CAD build for the part. Positions are in the model's coordinates, mm. A direction names the side the tool comes from. Give positions to 0.01 mm unless a question says otherwise; leave off trailing zeros. Write each loop counter-clockwise with the first axis right and the second up, starting at its lowest first coordinate (ties: lowest second). Pieces come first, ordered by that corner, then holes. Notation, with made-up numbers: (-14, 5.25) - (33, 5.25) arc R36 ccw to (33, 41.25) - close; hole circle Ø6 at (-5.5, -25.5). An arc over 180 degrees is marked (long way). Write item = value, one per line. Start each with the question number.
```python
from build123d import *

# Parameters (mm, degrees)
SKETCH3_OUTSIDE_W   = 136.718
SKETCH3_OUTSIDE_H   = 136.718
CUT_EXTRUDE2_DEPTH  = 5.463617
SKETCH4_W           = 9.6
SKETCH4_H           = 1.5
BOSS_EXTRUDE1_DEPTH = 6


with BuildPart() as part:
    # Sketch2 → Base-Revolve (revolve)
    with BuildSketch(Plane(origin=(0, 0, 0), x_dir=(0, 0, -1), z_dir=(1, 0, 0))):
        Polygon((-3.963615094, 52.5), (0, 44), (0, 0), (-1.5, 0), (-1.5, 44), (-5.463615094, 52.5), align=None)
    revolve(axis=Axis((0, 0, 0), (0, 0, 1)))

    # Sketch3 outside → Cut-Extrude2 (cut)
    # profile 1 of 2: a face of its own
    with BuildSketch(Plane.XY):
        Rectangle(SKETCH3_OUTSIDE_W, SKETCH3_OUTSIDE_H)
        with BuildLine():
            Line((-4.8, -43.737398185), (-4.8, -52.280110941))
            Line((-4.8, -52.280110941), (4.8, -52.280110941))
            Line((4.8, -52.280110941), (4.8, -43.737398185))
            ThreePointArc((4.8, -43.737398185), (34.907546973, -26.785502876), (43.489413898, 6.683627667))
            Line((43.489413898, 6.683627667), (51.741040776, 8.894644425))
            Line((51.741040776, 8.894644425), (49.256377943, 18.167532358))
            Line((49.256377943, 18.167532358), (41.004751065, 15.9565156))
            ThreePointArc((41.004751065, 15.9565156), (38.105117767, 22), (34.321123398, 27.532898298))
            Line((34.321123398, 27.532898298), (40.361733517, 33.573508418))
            Line((40.361733517, 33.573508418), (33.573508418, 40.361733517))
            Line((33.573508418, 40.361733517), (27.532898298, 34.321123398))
            ThreePointArc((27.532898298, 34.321123398), (22, 38.105117767), (15.9565156, 41.004751065))
            Line((15.9565156, 41.004751065), (18.167532358, 49.256377943))
            Line((18.167532358, 49.256377943), (8.894644425, 51.741040776))
            Line((8.894644425, 51.741040776), (6.683627667, 43.489413898))
            ThreePointArc((6.683627667, 43.489413898), (-34.907546973, 26.785502876), (-40.277697924, -17.711777154))
            Line((-40.277697924, -17.711777154), (-47.675904188, -21.983133532))
            Line((-47.675904188, -21.983133532), (-42.875904188, -30.296977409))
            Line((-42.875904188, -30.296977409), (-35.477697924, -26.025621031))
            ThreePointArc((-35.477697924, -26.025621031), (-31.112698372, -31.112698372), (-26.025621031, -35.477697924))
            Line((-26.025621031, -35.477697924), (-30.296977409, -42.875904188))
            Line((-30.296977409, -42.875904188), (-21.983133532, -47.675904188))
            Line((-21.983133532, -47.675904188), (-17.711777154, -40.277697924))
            ThreePointArc((-17.711777154, -40.277697924), (-11.388037985, -42.500736357), (-4.8, -43.737398185))
        make_face(mode=Mode.SUBTRACT)
    # profile 2 of 2: a face of its own
    with BuildSketch(Plane.XY):
        with BuildLine():
            Line((4.8, -34.164455213), (4.8, -30.5))
            Line((4.8, -30.5), (-4.8, -30.5))
            Line((-4.8, -30.5), (-4.8, -34.164455213))
            ThreePointArc((-4.8, -34.164455213), (0, 34.5), (4.8, -34.164455213))
        make_face()
    extrude(amount=CUT_EXTRUDE2_DEPTH, mode=Mode.SUBTRACT)

    # Sketch4 → Boss-Extrude1 (add)
    with BuildSketch(Plane.XY):
        with Locations((0, -31.25)):
            Rectangle(SKETCH4_W, SKETCH4_H)
    extrude(amount=BOSS_EXTRUDE1_DEPTH)


solid = part.part
```
1. Cut at D-D (x = -12). Give the cut face in (y, z).
2. Mould opens along Y. For faces 1 (the conical face through (-24.22, -41.8, 3.51)), 2 (the flat face through (-4.8, -31, 2)), 3 (the flat face through (3, -33, 0)), 4 (the flat face through (-19.857, -43.994, 2.921)) say: +Y half, -Y half, draft (parallel to the pull), parting line (faces both ways), or undercut.
3. Cut at B-B (x = 0). Give the cut face in (y, z), then the cut area to 3 significant figures.
4. Wall check: line 1 along X through (y, z) = (0, 0.45); line 2 along Z through (x, y) = (-42, -8.5); line 3 along Y through (x, z) = (0, 0.4). Give the ranges that are in metal, low to high.
5. Pin check, flat tips, straight feed: pin 1 Ø1.1 at (y, z) = (-31.5, 1.5) entering from -X; pin 2 Ø12 at (x, y) = (34.5, 30) entering from +Z; pin 3 Ø2 at (x, z) = (41.5, 1.5) entering from -Y. Stop position of each tip, or through.
6. Tool access for faces 5 (the flat face through (0, -32, 4)), 6 (the flat face through (30.57, 37.36, 2.92)), 7 (the flat face through (-43.96, -19.84, 2.72)), 8 (the cylindrical face through (-11.479, -42.476, 0.74)): list every direction of +Z, -Z, +X, -X, +Y, -Y with a clear straight run to the whole face (end or side of a thin tool).
7. Cut at A-A (y = 0). Give the cut face in (x, z), then the cut area to 3 significant figures.
8. Cut at C-C (z = 2.5). Give the cut face in (x, y).
Output:
q1.outline = (-42.33, 0) - (-32.35, 0) - (-32.35, 1.5) - (-42.33, 1.5) - close; (32.35, 0) - (42.33, 0) - (42.33, 1.5) - (32.35, 1.5) - close
q2.face_1 = +Y half
q2.face_2 = undercut
q2.face_3 = draft
q2.face_4 = -Y half
q3.outline = (-52.28, 3.86) - (-44, 0) - (-30.5, 0) - (-30.5, 6) - (-32, 6) - (-32, 1.5) - (-44, 1.5) - (-52.28, 5.36) - close; (34.5, 0) - (44, 0) - (44, 1.5) - (34.5, 1.5) - close
q3.area = 53.7 mm2
q4.line_1 = -44 to -34.5, 34.5 to 44
q4.line_2 = 0 to 1.5
q4.line_3 = -44.86 to -30.5, 34.5 to 44
q5.pin_1 = -31.27
q5.pin_2 = 5.1
q5.pin_3 = -17.2
q6.face_5 = +Z, +X, -X
q6.face_6 = +Z, -Z, +Y
q6.face_7 = +Z, -Z, -X
q6.face_8 = +Z, -Z, -Y
q7.outline = (-44, 0) - (-34.5, 0) - (-34.5, 1.5) - (-44, 1.5) - close; (34.5, 0) - (44, 0) - (44, 1.5) - (34.5, 1.5) - close
q7.area = 28.5 mm2
q8.outline = (-44.95, -20.41) arc R49.36 ccw to (-40.15, -28.72) - (-37.35, -27.1) arc R46.14 cw to (-42.15, -18.79) - close; (-28.72, -40.15) arc R49.36 ccw to (-20.41, -44.95) - (-18.79, -42.15) arc R46.14 cw to (-27.1, -37.35) - close; (-4.8, -49.13) arc R49.36 ccw to (4.8, -49.13) - (4.8, -45.89) arc R46.14 cw to (-4.8, -45.89) - close; (-4.8, -32) - (4.8, -32) - (4.8, -30.5) - (-4.8, -30.5) - close; (7.24, 45.57) arc R46.14 cw to (16.51, 43.09) - (17.35, 46.21) arc R49.36 ccw to (8.08, 48.7) - close; (29.06, 35.85) arc R46.14 cw to (35.85, 29.06) - (38.13, 31.34) arc R49.36 ccw to (31.34, 38.13) - close; (43.09, 16.51) arc R46.14 cw to (45.57, 7.24) - (48.7, 8.08) arc R49.36 ccw to (46.21, 17.35) - close
